Could you check a few things on this model? Use its own coordinates, in mm. Coordinates: 2 decimals unless noted, no trailing zeros. Write each loop counter-clockwise with the first axis right and the second up, starting at its lowest first coordinate (ties: lowest second). Pieces come first, ordered by that corner, then holes. Notation, with made-up numbers: M 79.5,51 L 96.5,51 A27 cw 96.5,72 Z; hole C 89.25,-15.75 d7. An arc over 180 degrees is marked long. Write item = value, one per line.
```python
from build123d import *

# Parameters (mm, degrees)
EXTRUDE_1_DEPTH         = 8
HOLE_WIZARD_M12_1_D     = 10.2
HOLE_WIZARD_M12_1_DEPTH = 29.25
HOLE_WIZARD_M12_1_TIP   = 3.064389157
SKETCH_5_R              = 10
CUT_EXTRUDE_1_DEPTH     = 8


with BuildPart() as part:
    # 草图1 → 凸台-拉伸1 (new body)
    with BuildSketch(Plane.XY):
        with BuildLine():
            Line((-73.159574468, 12.213789897), (-5.85106383, 26.870337773))
            ThreePointArc((-5.85106383, 26.870337773), (0, 27.5), (5.85106383, 26.870337773))
            Line((5.85106383, 26.870337773), (73.159574468, 12.213789897))
            ThreePointArc((73.159574468, 12.213789897), (83, 0), (73.159574468, -12.213789897))
            Line((73.159574468, -12.213789897), (5.85106383, -26.870337773))
            ThreePointArc((5.85106383, -26.870337773), (0, -27.5), (-5.85106383, -26.870337773))
            Line((-5.85106383, -26.870337773), (-73.159574468, -12.213789897))
            ThreePointArc((-73.159574468, -12.213789897), (-83, 0), (-73.159574468, 12.213789897))
        make_face()
    extrude(amount=EXTRUDE_1_DEPTH)

    # M12 螺纹孔1
    with Locations(Plane.XY.offset(8)):
        with Locations((-70.5, 0), (70.5, 0)):
            Hole(HOLE_WIZARD_M12_1_D / 2, depth=HOLE_WIZARD_M12_1_DEPTH)
            with Locations((0, 0, -(HOLE_WIZARD_M12_1_DEPTH + HOLE_WIZARD_M12_1_TIP / 2))):  # 118° drill point
                Cone(0, HOLE_WIZARD_M12_1_D / 2, HOLE_WIZARD_M12_1_TIP, mode=Mode.SUBTRACT)

    # 草图5 → 切除-拉伸1 (cut)
    with BuildSketch(Plane.XY.offset(8)):
        Circle(SKETCH_5_R)
    extrude(amount=-CUT_EXTRUDE_1_DEPTH, mode=Mode.SUBTRACT)


solid = part.part
```
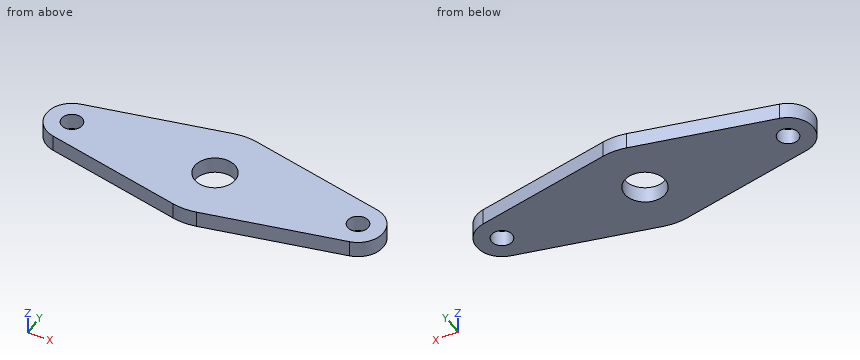
Item 1: I'm going to push flat-ended pins straight in: P1, Ø4, axis at y = -6.5, z = 6.5, coming from the +X side; P2, Ø8, axis at x = -70.5, y = 0, coming from the +Z side; P3, Ø1, axis at y = 1, z = 4.5, coming from the -X side; P4, Ø1, axis at x = 37.5, z = 4.5, coming from the +Y side. Where does each tip first touch, or does it pass through?
Numbers:
P1 = 82.16
P2 = through
P3 = -82.99
P4 = 20.09
Item 2: Imagine slicing it at B-B (z = 3.5). Write out the boundary of the cut face in (x, y).
Numbers:
outline = M -73.16,-12.21 L -5.85,-26.87 A27.5 ccw 5.85,-26.87 L 73.16,-12.21 A12.5 ccw 73.16,12.21 L 5.85,26.87 A27.5 ccw -5.85,26.87 L -73.16,12.21 A12.5 ccw Z; hole C -70.5,0 d10.2; hole C 0,0 d20; hole C 70.5,0 d10.2
Item 3: Imagine slicing it at A-A (y = 0). Write out the boundary of the cut face in (x, z).
Numbers:
outline = M -83,0 L -75.6,0 L -75.6,8 L -83,8 Z; M -65.4,0 L -10,0 L -10,8 L -65.4,8 Z; M 10,0 L 65.4,0 L 65.4,8 L 10,8 Z; M 75.6,0 L 83,0 L 83,8 L 75.6,8 Z
Item 4: Imagine slicing it at D-D (x = -22.5). Write out the boundary of the cut face in (y, z) (3 decimals).
Numbers:
outline = M -23.245,0 L 23.245,0 L 23.245,8 L -23.245,8 Z
Item 5: Imagine slicing it at C-C (x = 67). Write out the boundary of the cut face in (y, z).
Numbers:
outline = M -13.56,0 L -3.71,0 L -3.71,8 L -13.56,8 Z; M 3.71,0 L 13.56,0 L 13.56,8 L 3.71,8 Z
Item 6: If I drill on line 1 along Y through (x, z) = (0, 2); line 2 along X through (y, z) = (-4, 3.5); line 3 along Y through (x, z) = (53, 4.75), over which ranges is the centre line in solid material (lowest first)?
Numbers:
line_1 = -27.5 to -10, 10 to 27.5
line_2 = -82.34 to -73.66, -67.34 to -9.17, 9.17 to 67.34, 73.66 to 82.34
line_3 = -16.6 to 16.6
